```python
from build123d import *

# Parameters (mm, degrees)
SKETCH_1_W          = 45
SKETCH_1_H          = 40
EXTRUDE_1_DEPTH     = 10
CUT_EXTRUDE_1_DEPTH = 20


with BuildPart() as part:
    # 草图1 → 凸台-拉伸1 (new body)
    with BuildSketch(Plane(origin=(0, 0, 0), x_dir=(1, 0, 0), z_dir=(0, 1, 0))):
        Rectangle(SKETCH_1_W, SKETCH_1_H)
    extrude(amount=EXTRUDE_1_DEPTH)

    # 草图2 → 切除-拉伸1 (cut)
    with BuildSketch(Plane(origin=(0, 10, 0), x_dir=(1, 0, 0), z_dir=(0, 1, 0))):
        Polygon((22.5, 20), (-17.5, 20), (22.5, -15), align=None)
    extrude(amount=-CUT_EXTRUDE_1_DEPTH, mode=Mode.SUBTRACT)


solid = part.part
```
Verification items for the finished model (mm, model axes). Round coordinates to 2 decimals unless told otherwise and drop trailing zeros. Order: outer loops, then holes, each group sorted by start corner. A loop starts at its lowest first (then second) coordinate and runs counter-clockwise, first axis right, second up. Notation, with made-up numbers: (-22.5, 84.25) -> (26.5, 84.25) arc R17 ccw to (26.5, 96.25) -> close; hole circle Ø1 at (-3.5, 6.25). An arc over 180 degrees is marked (long way). Put each result on its own line as item: value. Start each with the question number.
(1) Section check C-C (z = -6). Enter the section's corners in (x, y).
(2) Section check B-B (x = -3.5). Enter the section's corners in (y, z).
(3) Material ranges on line 1 along X through (y, z) = (3, 6); line 2 along X through (y, z) = (9.25, -16.5); line 3 along Z through (x, y) = (2, 6.5), recorded low to high.
(4) Section check A-A (y = 2). Enter the section's corners in (x, z).
(5) Depth check by flat-ended pin: pin 1 Ø3 at (x, y) = (13.5, 2) entering from -Z. Enter the tip coordinate at first touch or a pass-through.
Completed:
1. outline: (-22.5, 0) -> (-1.5, 0) -> (-1.5, 10) -> (-22.5, 10) -> close
2. outline: (0, -7.75) -> (10, -7.75) -> (10, 20) -> (0, 20) -> close
3. line 1: x = -22.5 to 12.21
3. line 2: x = -22.5 to -13.5
3. line 3: z = -2.94 to 20
4. outline: (-22.5, -20) -> (-17.5, -20) -> (22.5, 15) -> (22.5, 20) -> (-22.5, 20) -> close
5. pin 1: stops at z = 5.81
